Verification items for the finished model (mm, model axes). A direction names the side the tool comes from. Give positions to 0.01 mm unless a question says otherwise; leave off trailing zeros. Write each loop counter-clockwise with the first axis right and the second up, starting at its lowest first coordinate (ties: lowest second). Pieces come first, ordered by that corner, then holes. Notation, with made-up numbers: (36, 69) -> (80, 69) arc R21 cw to (80, 102) -> close; hole circle Ø2 at (85, 13). An arc over 180 degrees is marked (long way). Use one line per item in the form item = value. Start each with the question number.
(1) Scan lines: L1, parallel to X at y = 294.5, z = 10.25; L2, parallel to Z at x = -47, y = 390.5; L3, parallel to X at y = 317, z = 6.25. Record each from-to range of solid material in increasing order.
(2) Section check C-C, the plane z = 18.75. Record the cut outline in (x, y), plus the area to 3 significant figures.
(3) Section check D-D, the plane y = 81. Record the cut outline in (x, z).
(4) Set-up check for faces 4 (the face through (144.78, 126.53, 12.32)), 5 (the face through (-16.012, 411.953, 0.986)): record each of +Z, -Z, +X, -X, +Y, -Y from which the full face is reachable in a straight line by a thin tool's end or side.
(5) Depth check by flat-ended pin: pin 1 Ø2 at (x, z) = (-123, 16.5) entering from +Y; pin 2 Ø6 at (y, z) = (209, 8) entering from +X; pin 3 Ø6 at (y, z) = (92.5, 20) entering from +X. Enter the tip coordinate at first touch or a pass-through.
(6) Section check A-A, the plane y = 290. Record the cut outline in (x, z).
(7) Section check B-B, the plane x = 0. Record the cut outline in (y, z), plus the area to 3 significant figures.
(8) Release check for a two-part mould opening along X. For faces 1 (the face through (-145.485, 130.123, 12.325)), 2 (the face through (-14.32, 399.064, 13.339)), 3 (the face through (36, 183, 25)) record: pulls with the +X half, pulls with the -X half, needs draft (parallel to the pull), parting line crosses it, or undercut.
from build123d import *

# Parameters (mm, degrees)
SKETCH1_R           = 110
BOSS_EXTRUDE1_DEPTH = 25
SKETCH2_R           = 123
SKETCH2_R_2         = 110
CUT_EXTRUDE2_DEPTH  = 2


with BuildPart() as part:
    # Sketch1 → Boss-Extrude1 (new body)
    with BuildSketch(Plane.XY):
        with BuildLine():
            Line((-120, 0), (120, 0))
            Line((120, 0), (170.2653156, 256.653751283))
            ThreePointArc((170.2653156, 256.653751283), (0, 463.5), (-170.2653156, 256.653751283))
            Line((-170.2653156, 256.653751283), (-120, 0))
        make_face()
        with Locations((0, 290)):
            Circle(SKETCH1_R, mode=Mode.SUBTRACT)
    extrude(amount=BOSS_EXTRUDE1_DEPTH)

    # Sketch2 → Cut-Extrude2 (cut)
    with BuildSketch(Plane.XY):
        with Locations((0, 290)):
            Circle(SKETCH2_R)
        with Locations((0, 290)):
            Circle(SKETCH2_R_2, mode=Mode.SUBTRACT)
    extrude(amount=CUT_EXTRUDE2_DEPTH, mode=Mode.SUBTRACT)


solid = part.part
Completed:
q1.L1 = -173.44 to -109.91, 109.91 to 173.44
q1.L2 = 2 to 25
q1.L3 = -171.39 to -106.63, 106.63 to 171.39
q2.outline = (-170.27, 256.65) -> (-120, 0) -> (120, 0) -> (170.27, 256.65) arc R173.5 ccw (long way) to start; hole circle Ø220 at (0, 290)
q2.area = 95,300 mm²
q3.outline = (-135.86, 0) -> (135.86, 0) -> (135.86, 25) -> (-135.86, 25) -> close
q4.face_4 = +Z, -Z, +X, -Y
q4.face_5 = -Z
q5.pin_1 = 413.36
q5.pin_2 = 161.52
q5.pin_3 = 138.7
q6.outline = (-173.5, 0) -> (-123, 0) -> (-123, 2) -> (-110, 2) -> (-110, 25) -> (-173.5, 25) -> close; (110, 2) -> (123, 2) -> (123, 0) -> (173.5, 0) -> (173.5, 25) -> (110, 25) -> close
q7.outline = (0, 0) -> (167, 0) -> (167, 2) -> (180, 2) -> (180, 25) -> (0, 25) -> close; (400, 2) -> (413, 2) -> (413, 0) -> (463.5, 0) -> (463.5, 25) -> (400, 25) -> close
q7.area = 6,040 mm²
q8.face_1 = pulls with the -X half
q8.face_2 = undercut
q8.face_3 = needs draft
